```python
from build123d import *

# Parameters (mm, degrees)
SKETCH1_R           = 1.179493096
BOSS_EXTRUDE1_DEPTH = 59.73181499
SKETCH2_R           = 5.417808654
BOSS_EXTRUDE2_DEPTH = 5


with BuildPart() as part:
    # Sketch1 → Boss-Extrude1 (new body)
    with BuildSketch(Plane.XY):
        with Locations((-29.791335202, -6.219759883)):
            Circle(SKETCH1_R)
    extrude(amount=-BOSS_EXTRUDE1_DEPTH)

    # Sketch2 → Boss-Extrude2 (add)
    with BuildSketch(Plane.XY):
        with Locations((-29.791335202, -6.219759883)):
            Circle(SKETCH2_R)
    boss_extrude2 = extrude(amount=BOSS_EXTRUDE2_DEPTH)

    # Mirror1: Boss-Extrude2 across plane
    add(boss_extrude2.mirror(Plane.XY.offset(-29.865907495)))

    # Sketch4 → Cut-Revolve2 (revolve, cut)
    with BuildSketch(Plane(origin=(0, -6.219759883, 0), x_dir=(0, 0, -1), z_dir=(0, 1, 0)), mode=Mode.PRIVATE) as cut_revolve2_sk:
        Polygon((-4.042100794, 35.209143856), (-3.05057693, 34.217619991), (-1.94942307, 34.217619991), (-0.957899206, 35.209143856), align=None)
        Polygon((60.689714196, 35.209143856), (61.68123806, 34.217619991), (62.78239192, 34.217619991), (63.773915784, 35.209143856), align=None)
    revolve(cut_revolve2_sk.sketch.rotate(Axis((-29.791335202, -6.219759883, 5), (0, 0, -1)), 180), axis=Axis((-29.791335202, -6.219759883, 5), (0, 0, -1)), mode=Mode.SUBTRACT)


solid = part.part
```
CAD build for the part. Positions are in the model's coordinates, mm. A direction names the side the tool comes from. Give positions to 0.01 mm unless a question says otherwise; leave off trailing zeros. Write each loop counter-clockwise with the first axis right and the second up, starting at its lowest first coordinate (ties: lowest second). Pieces come first, ordered by that corner, then holes. Notation, with made-up numbers: (-34.75, -22) -> (-3.75, -22) arc R10 ccw to (-3.75, -3) -> close; hole circle Ø1 at (13.5, -24.75). An arc over 180 degrees is marked (long way). Write each question's results on one line, items separated by ' | '.
1. Wall check: probe 1 along Z at (x, y) = (-31.25, -7.5); probe 2 along Z at (x, y) = (-25.5, -9.25); probe 3 along Z at (x, y) = (-32.25, -2.5) (3 decimals). Give the ranges that are in metal, low to high. Write a range as [from, to].
Geometry check:
probe 1: [-64.73, -59.73], [0, 5] | probe 2: [-64.73, -63.61], [-60.85, -59.73], [0, 1.12], [3.88, 5] | probe 3: [-64.732, -62.815], [-61.649, -59.732], [0, 1.917], [3.083, 5]
2. Two-plate mould, pull along Z, no slides. Class faces 1 (the cylindrical face through (-25.703, -4.524, 2.492)), 2 (the flat face through (-30, -6, -64.732)), 3 (the cylindrical face through (-35.204, -5.982, 0.472)): pulls with the +Z half, pulls with the -Z half, needs draft (parallel to the pull), parting line crosses it, or undercut.
Geometry check:
face 1: undercut | face 2: pulls with the -Z half | face 3: needs draft
3. Which spindle directions (+Z, -Z, +X, -X, +Y, -Y) get a long thin tool onto all of the face, cutting with end or side? Do faces 4 (the cylindrical face through (-25.703, -4.524, -62.24)), 5 (the flat face through (-30, -6, 5)). Say none if no direction does.
Geometry check:
face 4: none | face 5: +Z, +X, -X, +Y, -Y
4. Drop flat-ended pins along their axis: P1, Ø4, axis at y = -6.5, z = -42, coming from the +X side; P2, Ø4, axis at y = -7.5, z = -37.5, coming from the -X side; P3, Ø6, axis at x = -30.5, z = -36.5, coming from the +Y side. Give the stop position or say it passes through.
Geometry check:
P1: x = -28.61 | P2: x = -30.97 | P3: y = -5.04
5. Cut at A-A, the plane z = -11. Write the cut outline in (x, y), then the cut area to 3 significant figures.
Geometry check:
outline: circle Ø2.36 at (-29.79, -6.22) | area: 4.37 mm²
